```python
from build123d import *

# Parameters (mm, degrees)
INVERTED_U_FORK_BODY_DEPTH    = 60
TOP_COLLAR_BOSS_SKETCH_R      = 20
TOP_COLLAR_BOSS_SKETCH_R_2    = 12.5
TOP_COLLAR_BOSS_DEPTH         = 5
COLLAR_START                  = -50
COLLAR_BORE_SKETCH_R          = 12.5
COLLAR_BORE_25_DEPTH          = 50
LEG_BLEND_FILLET_R20_A_R      = 20
LEG_BLEND_FILLET_R20_B_R      = 20
LEG_PIN_HOLE_SKETCH_R         = 10
LEG_PIN_HOLES_20_DEPTH        = 200
SIDE_BOSS_A_SKETCH_R          = 20
SIDE_BOSS_A_SKETCH_R_2        = 10
SIDE_BOSS_A_DEPTH             = 50
SIDE_START                    = -50
SIDE_BOSS_B_SKETCH_R          = 20
SIDE_BOSS_B_SKETCH_R_2        = 10
SIDE_BOSS_B_DEPTH             = 50
SIDE_START_2                  = -180
SIDE_BOSS_CROSS_BORE_SKETCH_R = 10
SIDE_BOSS_CROSS_BORE_20_DEPTH = 180
WEB_RIB_DEPTH                 = 7.5


with BuildPart() as part:
    # Fork Profile Sketch → Inverted U Fork Body (new body)
    with BuildSketch(Plane.XY):
        with BuildLine():
            Line((-25.320668346, 110.01352712), (-25.320668346, 141.01352712))
            ThreePointArc((-25.320668346, 141.01352712), (-24.734881908, 142.427740683), (-23.320668346, 143.01352712))
            Line((-23.320668346, 143.01352712), (22.679331654, 143.01352712))
            ThreePointArc((22.679331654, 143.01352712), (24.093545217, 142.427740683), (24.679331654, 141.01352712))
            Line((24.679331654, 141.01352712), (24.679331654, 110.01352712))
            Line((24.679331654, 110.01352712), (60, 52))
            Line((60, 52), (60, 0))
            Line((60, 0), (80, 0))
            Line((80, 0), (80, 52))
            Line((80, 52), (44.679331654, 110.01352712))
            Line((44.679331654, 110.01352712), (44.679331654, 153))
            ThreePointArc((44.679331654, 153), (41.750399466, 160.071067812), (34.679331654, 163))
            Line((34.679331654, 163), (24.679331654, 163))
            Line((24.679331654, 163), (24.679331654, 172))
            Line((24.679331654, 172), (10, 172))
            Line((10, 172), (-10, 172))
            Line((-10, 172), (-25.320668346, 172))
            Line((-25.320668346, 172), (-25.320668346, 163))
            Line((-25.320668346, 163), (-35.320668346, 163))
            ThreePointArc((-35.320668346, 163), (-42.391736158, 160.071067812), (-45.320668346, 153))
            Line((-45.320668346, 153), (-45.320668346, 110.01352712))
            Line((-45.320668346, 110.01352712), (-80, 52))
            Line((-80, 52), (-80, 0))
            Line((-80, 0), (-60, 0))
            Line((-60, 0), (-60, 52))
            Line((-60, 52), (-25.320668346, 110.01352712))
        make_face()
    extrude(amount=INVERTED_U_FORK_BODY_DEPTH)

    # Top Collar Boss Sketch → Top Collar Boss (add)
    with BuildSketch(Plane(origin=(0, 172, 0), x_dir=(1, 0, 0), z_dir=(0, 1, 0))):
        with Locations(Location((0, -30, 0), (0, 0, 270))):
            Circle(TOP_COLLAR_BOSS_SKETCH_R)
        with Locations(Location((0, -30, 0), (0, 0, 270))):
            Circle(TOP_COLLAR_BOSS_SKETCH_R_2, mode=Mode.SUBTRACT)
    extrude(amount=TOP_COLLAR_BOSS_DEPTH)

    # Collar Bore Sketch → Collar Bore Ø25 (cut)
    with BuildSketch(Plane(origin=(0, 172, 0), x_dir=(1, 0, 0), z_dir=(0, 1, 0)).offset(COLLAR_START)):
        with Locations(Location((0, -30, 0), (0, 0, 270))):
            Circle(COLLAR_BORE_SKETCH_R)
    extrude(amount=COLLAR_BORE_25_DEPTH, mode=Mode.SUBTRACT)

    # Leg Blend Fillet R20 A
    leg_blend_fillet_r20_a_edges = [part.edges().sort_by_distance(p)[0] for p in [
        (-80, 52, 30),
    ]]
    fillet(leg_blend_fillet_r20_a_edges, radius=LEG_BLEND_FILLET_R20_A_R)

    # Leg Blend Fillet R20 B
    leg_blend_fillet_r20_b_edges = [part.edges().sort_by_distance(p)[0] for p in [
        (80, 52, 30),
    ]]
    fillet(leg_blend_fillet_r20_b_edges, radius=LEG_BLEND_FILLET_R20_B_R)

    # Leg Pin Hole Sketch → Leg Pin Holes Ø20 (cut)
    with BuildSketch(Plane.ZY.offset(80)):
        with Locations((30, 23.238954536)):
            Circle(LEG_PIN_HOLE_SKETCH_R)
    extrude(amount=-LEG_PIN_HOLES_20_DEPTH, mode=Mode.SUBTRACT)

    # Side Boss A Sketch → Side Boss A (add)
    with BuildSketch(Plane(origin=(30, 0, 0), x_dir=(0, 0, -1), z_dir=(1, 0, 0))):
        with Locations(Location((-30, 125.01352712, 0), (0, 0, 228.590377891))):
            Circle(SIDE_BOSS_A_SKETCH_R)
        with Locations((-30, 125.01352712)):
            Circle(SIDE_BOSS_A_SKETCH_R_2, mode=Mode.SUBTRACT)
    extrude(amount=SIDE_BOSS_A_DEPTH)

    # Side Boss B Sketch → Side Boss B (add)
    with BuildSketch(Plane(origin=(-30, 0, 0), x_dir=(0, 0, -1), z_dir=(1, 0, 0)).offset(SIDE_START)):
        with Locations(Location((-30, 125.01352712, 0), (0, 0, 228.590377891))):
            Circle(SIDE_BOSS_B_SKETCH_R)
        with Locations((-30, 125.01352712)):
            Circle(SIDE_BOSS_B_SKETCH_R_2, mode=Mode.SUBTRACT)
    extrude(amount=SIDE_BOSS_B_DEPTH)

    # Side Boss Cross Bore Sketch → Side Boss Cross Bore Ø20 (cut)
    with BuildSketch(Plane(origin=(44.679331654, 0, 0), x_dir=(0, 0, -1), z_dir=(1, 0, 0)).offset(SIDE_START_2)):
        with Locations(Location((-30, 125.01352712, 0), (0, 0, 90))):
            Circle(SIDE_BOSS_CROSS_BORE_SKETCH_R)
    extrude(amount=SIDE_BOSS_CROSS_BORE_20_DEPTH, mode=Mode.SUBTRACT)

    # Web Rib Sketch → Web Rib (add, symmetric)
    with BuildSketch(Plane.XY.offset(30)):
        Polygon((-45.320668346, 110.01352712), (-80, 110.01352712), (-80, 46.477909073), align=None)
        Polygon((44.679331654, 110.01352712), (80, 110.01352712), (80, 46.390582944), align=None)
    extrude(amount=WEB_RIB_DEPTH, both=True)


solid = part.part
```
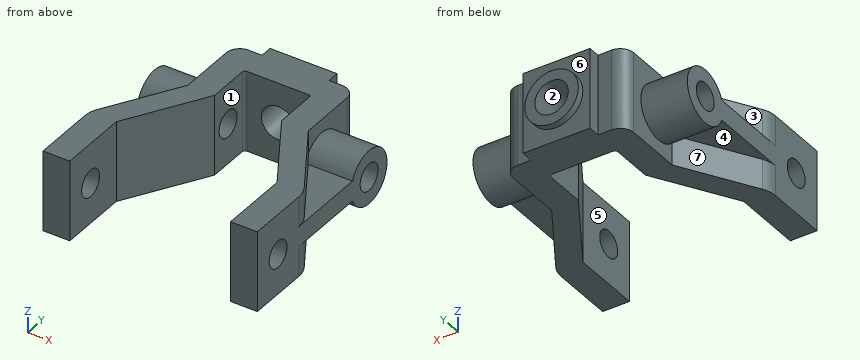
Can you work these out from the model? Positions are in its coordinate system, mm. Face numbers are marked on the shaded views. A direction names the side the tool comes from. Coordinates: 2 decimals unless noted, no trailing zeros. Loops run counter-clockwise (first coordinate to the right, second up) from the corner with the lowest first, then second, coordinate; pieces in that order, holes last. Notation, with made-up numbers: (22, 27) -> (66, 27) arc R27 cw to (66, 62) -> close; hole circle Ø6 at (42, -22.75). An arc over 180 degrees is marked (long way). Put each result on its own line as item: value. Start each with the question number.
Q1. I want a section at A-A (x = 0). Write out the boundary of the cut face in (y, z), plus the area to 3 significant figures.
Q2. I want a section at D-D (y = 149.5). Write out the boundary of the cut face in (x, z).
Q3. If I drill on line 1 (X direction, y = 112, z = 44); line 2 (X direction, y = 129.5, z = 53); line 3 (Z direction, x = -32.5, y = 130), over which ranges is the centre line in solid material (lowest first)? Write a range as [from, to].
Q4. I'm going to push flat-ended pins straight in: P1, Ø5, axis at y = 65.5, z = 46, coming from the -X side; P2, Ø4, axis at y = 71, z = 47.5, coming from the -X side; P3, Ø4, axis at y = 52.5, z = 42, coming from the -X side. Where does each tip first touch, or does it pass through?
Q5. I want a section at B-B (y = 101). Write out the boundary of the cut face in (x, z), plus the area to 3 significant figures.
Q6. Thinking about a two-plate mould opening in Y: for the marked faces 5, 6 and 7, which applies, pulls with the +Y half, pulls with the -Y half, needs draft (parallel to the pull), parting line crosses it, or undercut?
Q7. For the marked faces 1, 2, 3 and 4, which set-ups out of +Z, -Z, +X, -X, +Y, -Y let a thin tool reach every point of the face, with its end or its side?
Taken from the geometry:
1. outline: (143.01, 0) -> (172, 0) -> (172, 10) -> (177, 10) -> (177, 17.5) -> (143.01, 17.5) -> close; (143.01, 42.5) -> (177, 42.5) -> (177, 50) -> (172, 50) -> (172, 60) -> (143.01, 60) -> close
1. area: 1,090 mm2
2. outline: (-45.32, 0) -> (44.68, 0) -> (44.68, 60) -> (-45.32, 60) -> close; hole circle Ø25 at (0, 30)
3. line 1: x = [-80, -25.32], [24.68, 80]
3. line 2: x = [-45.32, -25.32], [24.68, 44.68]
3. line 3: z = [0, 21.33], [38.67, 60]
4. P1: stops at x = -73.42
4. P2: stops at x = -69.84
4. P3: stops at x = -79.59
5. outline: (-80, 22.5) -> (-50.71, 22.5) -> (-50.71, 0) -> (-30.71, 0) -> (-30.71, 60) -> (-50.71, 60) -> (-50.71, 37.5) -> (-80, 37.5) -> close; (30.17, 0) -> (50.17, 0) -> (50.17, 22.5) -> (80, 22.5) -> (80, 37.5) -> (50.17, 37.5) -> (50.17, 60) -> (30.17, 60) -> close
5. area: 3,290 mm2
6. face 5: needs draft
6. face 6: pulls with the +Y half
6. face 7: undercut
7. face 1: +Z, -Z, -Y
7. face 2: +Y, -Y
7. face 3: +Z, -X
7. face 4: -Z, -X
